```python
from build123d import *

# Parameters (mm, degrees)
SKETCH1_W          = 32.173358544
SKETCH1_H          = 32.173358544
BASE_EXTRUDE_DEPTH = 15
SKETCH4_OUTSIDE_W  = 164.92
SKETCH4_OUTSIDE_H  = 164.92
SKETCH4_OUTSIDE_R  = 16.086679272
CUT_EXTRUDE1_DEPTH = 28.25
CUT_EXTRUDE1_DRAFT = -65
FILLET1_R          = 0.8


with BuildPart() as part:
    # Sketch1 → Base-Extrude (new body)
    with BuildSketch(Plane.XY):
        Rectangle(SKETCH1_W, SKETCH1_H)
    extrude(amount=BASE_EXTRUDE_DEPTH)


with BuildPart() as cut_extrude1_tool:
    # Sketch4 outside → Cut-Extrude1 (with draft: the straight prism first)
    with BuildSketch(Plane.XY.offset(15)):
        Rectangle(SKETCH4_OUTSIDE_W, SKETCH4_OUTSIDE_H)
        Circle(SKETCH4_OUTSIDE_R, mode=Mode.SUBTRACT)
    extrude(amount=-CUT_EXTRUDE1_DEPTH)
    # Cut-Extrude1: the draft: its side faces are tilted about the plane it starts from
    cut_extrude1_sides = [cut_extrude1_tool.faces().sort_by_distance(p)[0] for p in [
        (0, -82.46, 0.875),
        (82.46, 0, 0.875),
        (0, 82.46, 0.875),
        (-82.46, 0, 0.875),
        (-16.086679272, 0, 0.875),
    ]]
    draft(cut_extrude1_sides, Plane.XY.offset(15), CUT_EXTRUDE1_DRAFT)


with BuildPart() as part_1:
    add(part.part)

    # Cut-Extrude1: cut by cut_extrude1_tool
    add(cut_extrude1_tool.part, mode=Mode.SUBTRACT)

    # Sketch2 → Boss-Revolve1 (revolve)
    with BuildSketch(Plane(origin=(0, 0, 0), x_dir=(1, 0, 0), z_dir=(0, 1, 0)), mode=Mode.PRIVATE) as boss_revolve1_sk:
        Polygon((0, 0), (10.5, 0), (10.5, 87.401923789), (12, 90), (12, 150), (0, 150), align=None)
    revolve(boss_revolve1_sk.sketch.rotate(Axis((0, 0, -150), (0, 0, 1)), 180), axis=Axis((0, 0, -150), (0, 0, 1)))

    # Fillet1
    fillet1_edges = [part_1.edges().sort_by_distance(p)[0] for p in [
        (10.5, 0, 0),
    ]]
    fillet(fillet1_edges, radius=FILLET1_R)

    # Sketch3 → Cut-Revolve1 (revolve, cut)
    with BuildSketch(Plane(origin=(0, 0, 0), x_dir=(1, 0, 0), z_dir=(0, 1, 0))):
        Polygon((9.402, 150), (12, 151.499955999), (12, 148.500044001), align=None)
    revolve(axis=Axis((0, 0, 0), (0, 0, -1)), mode=Mode.SUBTRACT)


solid = part_1.part
```
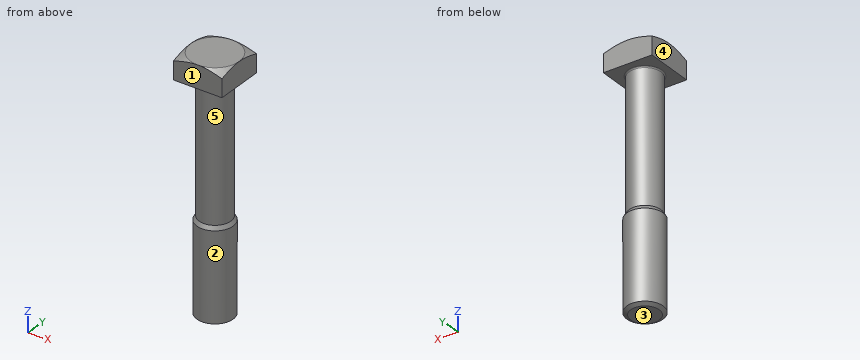
Work out the finished part from the listing and answer in its coordinate system (mm). Face numbers are marked on the shaded views. A direction names the side the tool comes from. Round coordinates to 2 decimals unless told otherwise and drop trailing zeros. Write each loop counter-clockwise with the first axis right and the second up, starting at its lowest first coordinate (ties: lowest second). Pieces come first, ordered by that corner, then holes. Notation, with made-up numbers: (52.25, 37.5) - (92.25, 37.5) arc R22 ccw to (92.25, 75.5) - close; hole circle Ø9 at (17, -29.5). An arc over 180 degrees is marked (long way). Return JSON: item names as keys, results as strings. Group by question number.
Q1. The part is cut by section A-A on z = -95. Write down the section's boundary in (x, y), then the cut area to 3 significant figures.
Q2. Each of these flat-tipped pins is pushed along its axis until it touches: pin 1 Ø2 at (x, y) = (11.5, 10) entering from -Z; pin 2 Ø8 at (x, z) = (-5, -121) entering from +Y; pin 3 Ø1.5 at (y, z) = (-3, -73) entering from -X. Where does it stop, or does it pass through?
Q3. Find the intervals of material crossed by L1, parallel to Y at x = -0.5, z = -135; L2, parallel to Z at x = -9.5, y = -9; L3, parallel to Z at x = -10.5, y = 3, in increasing order.
Q4. The part is cut by section B-B on z = -16. Write down the section's boundary in (x, y).
Q5. The mould has two halves that part along Z. Classify the marked faces 3, 4 and 5: released by +Z, released by -Z, zero draft, split by the parting line, or undercut.
Q6. For the marked faces 1 and 2, determine the directions among +Z, -Z, +X, -X, +Y, -Y from which every point of the face is accessible in a straight line to the end or side of a thin tool.
Solved:
{
 "1": {"outline": "circle Ø24 at (0, 0)", "area": "452 mm²"},
 "2": {"pin 1": "z = 0", "pin 2": "y = 11.96", "pin 3": "x = -10.26"},
 "3": {"L1": "-11.99 to 11.99", "L2": "0 to 15", "L3": "-149.12 to -88.13, -0.1 to 15"},
 "4": {"outline": "circle Ø21 at (0, 0)"},
 "5": {"face 3": "released by -Z", "face 4": "zero draft", "face 5": "undercut"},
 "6": {"face 1": "+Z, -Z, +X, -X, -Y", "face 2": "-Z"}
}
